Could you check a few things on this model? Use its own coordinates, in mm. Face numbers are marked on the shaded views. Round coordinates to 2 decimals unless told otherwise and drop trailing zeros. Write each loop counter-clockwise with the first axis right and the second up, starting at its lowest first coordinate (ties: lowest second). Pieces come first, ordered by that corner, then holes. Notation, with made-up numbers: M 46,32 L 75,32 A23 cw 75,47 Z; hole C 26.25,5 d6. An arc over 180 degrees is marked long. One line per item, written item: value. Start each with the question number.
(1) I want a section at C-C on z = -26. Please give me the cut outline in (x, y).
(2) I'm going to push flat-ended pins straight in: pin 1 Ø5.5 at (x, y) = (60, 0) entering from -Z; pin 2 Ø5 at (y, z) = (-0.5, -39) entering from +X; pin 3 Ø1.5 at (y, z) = (3.5, -37.5) entering from +X; pin 4 Ø12 at (x, z) = (26, -26) entering from -Y. Where does each tip first touch, or does it pass through?
(3) If I drill on L1, parallel to X at y = 0, z = -5; L2, parallel to Y at x = 20, z = -8; L3, parallel to X at y = 0, z = -9.5, over which ranges is the centre line in solid material (lowest first)?
(4) I want a section at B-B on x = 26. Please give me the cut outline in (y, z).
(5) I want a section at A-A on y = 3.5. Please give me the cut outline in (x, z).
(6) I want a section at D-D on x = 49. Please give me the cut outline in (y, z).
(7) Thinking about a two-plate mould opening in Z: for the marked faces 1, 2, 3 and 4, which applies, released by +Z, released by -Z, zero draft, split by the parting line, or undercut?
```python
from build123d import *

# Parameters (mm, degrees)
EXTRUDE_1_DEPTH        = 5
CHAMFER_1_SIZE         = 2
HOLE_WIZARD_M5_1_D     = 4.2
HOLE_WIZARD_M5_1_DEPTH = 12.4
HOLE_WIZARD_M5_1_TIP   = 1.2618073
HOLE_WIZARD_M5_2_D     = 4.2
HOLE_WIZARD_M5_2_DEPTH = 12.4
HOLE_WIZARD_M5_2_TIP   = 1.2618073
SKETCH_6_R             = 10
CUT_EXTRUDE_1_DEPTH    = 100.498743711
CHAMFER_2_SIZE         = 0.5


with BuildPart() as part:
    # 草图1 → 凸台-拉伸1 (new, symmetric)
    with BuildSketch(Plane(origin=(0, 0, 0), x_dir=(1, 0, 0), z_dir=(0, 1, 0))):
        Polygon((0, 0), (0, 70), (5, 70), (70, 5), (70, 0), align=None)
    extrude(amount=EXTRUDE_1_DEPTH, both=True)

    # 倒角1
    chamfer_1_edges = [part.edges().sort_by_distance(p)[0] for p in [
        (0, 0, 0),
    ]]
    chamfer(chamfer_1_edges, length=CHAMFER_1_SIZE)

    # M5 螺纹孔1
    with Locations(Plane.XY):
        with Locations((60, 0), (20, 0)):
            Hole(HOLE_WIZARD_M5_1_D / 2, depth=HOLE_WIZARD_M5_1_DEPTH)
            with Locations((0, 0, -(HOLE_WIZARD_M5_1_DEPTH + HOLE_WIZARD_M5_1_TIP / 2))):  # 118° drill point
                Cone(0, HOLE_WIZARD_M5_1_D / 2, HOLE_WIZARD_M5_1_TIP, mode=Mode.SUBTRACT)

    # M5 螺纹孔2
    with Locations(Plane.ZY):
        with Locations((-19.054479799, 0), (-59.054479799, 0)):
            Hole(HOLE_WIZARD_M5_2_D / 2, depth=HOLE_WIZARD_M5_2_DEPTH)
            with Locations((0, 0, -(HOLE_WIZARD_M5_2_DEPTH + HOLE_WIZARD_M5_2_TIP / 2))):  # 118° drill point
                Cone(0, HOLE_WIZARD_M5_2_D / 2, HOLE_WIZARD_M5_2_TIP, mode=Mode.SUBTRACT)

    # 草图6 → 切除-拉伸1 (cut, through all)
    with BuildSketch(Plane.XZ.offset(5)):
        with Locations(Location((26, -26, 0), (0, 0, 270))):
            Circle(SKETCH_6_R)
    extrude(amount=-CUT_EXTRUDE_1_DEPTH, mode=Mode.SUBTRACT)

    # 倒角2
    chamfer_2_edges = [part.edges().sort_by_distance(p)[0] for p in [
        (37.5, 5, -37.5),
        (2.5, 5, -70),
        (36, -5, 0),
        (0, 5, -36),
        (36, 5, 0),
        (1, -5, -1),
        (1, 5, -1),
        (26, 5, -16),
        (26, -5, -16),
        (0, -5, -36),
        (2.5, -5, -70),
        (37.5, -5, -37.5),
        (70, -5, -2.5),
        (70, 5, -2.5),
    ]]
    chamfer(chamfer_2_edges, length=CHAMFER_2_SIZE)


solid = part.part
```
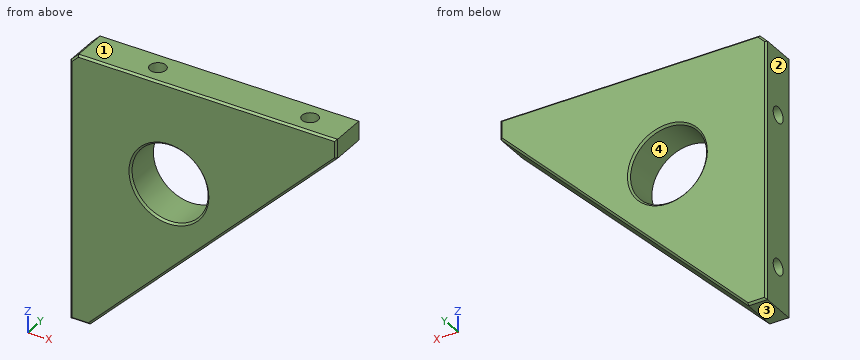
Found:
1. outline: M 0,-4.5 L 0.5,-5 L 15.5,-5 L 16,-4.5 L 16,4.5 L 15.5,5 L 0.5,5 L 0,4.5 Z; M 36,-4.5 L 36.5,-5 L 48.29,-5 L 49,-4.5 L 49,4.5 L 48.29,5 L 36.5,5 L 36,4.5 Z
2. pin 1: stops at z = -17.75
2. pin 2: stops at x = 38.5
2. pin 3: stops at x = 38.25
2. pin 4: passes through
3. L1: x = 0 to 17.9, 22.1 to 57.9, 62.1 to 70
3. L2: y = -5 to -2.1, 2.1 to 5
3. L3: x = 0 to 17.9, 22.1 to 57.9, 62.1 to 65.5
4. outline: M -5,-48.29 L -4.5,-49 L 4.5,-49 L 5,-48.29 L 5,-36.5 L 4.5,-36 L -4.5,-36 L -5,-36.5 Z; M -5,-15.5 L -4.5,-16 L 4.5,-16 L 5,-15.5 L 5,-0.5 L 4.5,0 L -4.5,0 L -5,-0.5 Z
5. outline: M 0,-70 L 5,-70 L 70,-5 L 70,0 L 2,0 L 0,-2 Z; hole C 26,-26 d20
6. outline: M -5,-25.29 L -4.5,-26 L 4.5,-26 L 5,-25.29 L 5,-0.5 L 4.5,0 L -4.5,0 L -5,-0.5 Z
7. face 1: released by +Z
7. face 2: zero draft
7. face 3: released by -Z
7. face 4: undercut
